from build123d import *

# Parameters (mm, degrees)
CHAMFER_1_SIZE           = 2
CUT_EXTRUDE_1_DEPTH      = 31
CUT_EXTRUDE_1_DEPTH_BACK = 20
SKETCH_2_W               = 91.624519514
SKETCH_2_H               = 25.767863676
HOLE_WIZARD_M10_1_D      = 8.5
HOLE_WIZARD_M10_1_DEPTH  = 27.5
HOLE_WIZARD_M10_1_TIP    = 2.553657631
CHAMFER_3_SIZE           = 1


with BuildPart() as part:
    # 草图1 → 旋转2 (revolve)
    with BuildSketch(Plane.XY):
        Polygon((0, 0), (0, 10), (23, 10), (23, 12.5), (120, 12.5), (120, 0), align=None)
    revolve(axis=Axis((120, 0, 0), (-1, 0, 0)))

    # 倒角1
    chamfer_1_edges = [part.edges().sort_by_distance(p)[0] for p in [
        (120, -12.5, 0),
        (0, -10, 0),
    ]]
    chamfer(chamfer_1_edges, length=CHAMFER_1_SIZE)

    # 草图2 → 切除-拉伸1 (cut, two sides: drawn at the far end of the back side and taken through both)
    with BuildSketch(Plane(origin=(0, 0, 0), x_dir=(1, 0, 0), z_dir=(0, 1, 0)).offset(-CUT_EXTRUDE_1_DEPTH_BACK)):
        with Locations((80.812259757, -17.883931838)):
            Rectangle(SKETCH_2_W, SKETCH_2_H)
    extrude(amount=CUT_EXTRUDE_1_DEPTH + CUT_EXTRUDE_1_DEPTH_BACK, mode=Mode.SUBTRACT)

    # M10 螺纹孔1
    with Locations(Plane.XY.offset(5)):
        with Locations((61, 0), (101, 0)):
            Hole(HOLE_WIZARD_M10_1_D / 2, depth=HOLE_WIZARD_M10_1_DEPTH)
            with Locations((0, 0, -(HOLE_WIZARD_M10_1_DEPTH + HOLE_WIZARD_M10_1_TIP / 2))):  # 118° drill point
                Cone(0, HOLE_WIZARD_M10_1_D / 2, HOLE_WIZARD_M10_1_TIP, mode=Mode.SUBTRACT)

    # 倒角3
    chamfer_3_edges = [part.edges().sort_by_distance(p)[0] for p in [
        (105.25, 0, 5),
        (65.25, 0, 5),
    ]]
    chamfer(chamfer_3_edges, length=CHAMFER_3_SIZE)


solid = part.part
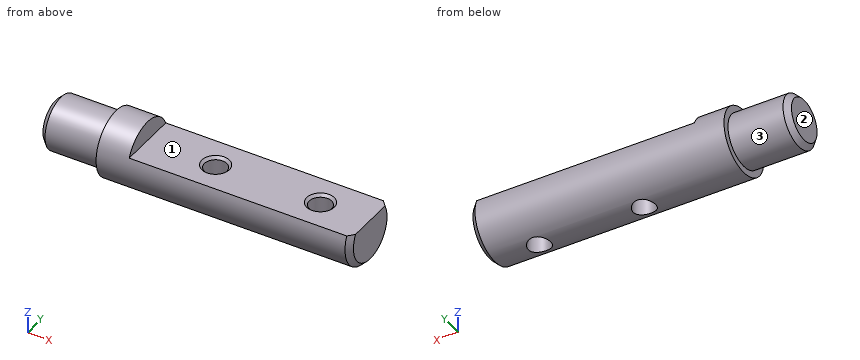
Design review of the part built by this model. Coordinates are the model's own, in mm. Face numbers are marked on the shaded views. Round coordinates to 2 decimals unless told otherwise and drop trailing zeros. Write each loop counter-clockwise with the first axis right and the second up, starting at its lowest first coordinate (ties: lowest second). Pieces come first, ordered by that corner, then holes. Notation, with made-up numbers: (-1, 15) - (28, 15) arc R30 ccw to (28, 46) - close; hole circle Ø2 at (62, 6). An arc over 180 degrees is marked (long way). Return JSON: item names as keys, results as strings. Group by question number.
Item 1: We need section D-D on x = 37.5. Write out the cut boundary in (y, z), and give its area (3 significant figures).
Item 2: We need section C-C on x = 61. Write out the cut boundary in (y, z).
Item 3: We need section B-B on y = 0. Write out the cut boundary in (x, z).
Item 4: The part is to be moulded in two halves that separate along Z. For the marked faces 1, 2 and 3, say which applies: pulls with the +Z half, pulls with the -Z half, needs draft (parallel to the pull), parting line crosses it, or undercut.
Item 5: We need section A-A on z = 0. Write out the cut boundary in (x, y).
Item 6: For probe 1 along X at (y, z) = (0, -5); probe 2 along Y at (x, z) = (101, -7.5); probe 3 along X at (y, z) = (-3.5, -2.75), list the stretches that pass through material, from the lowest coordinate up. Write a range as [from, to].
Item 7: Insertion check: P1, Ø1.5, axis at x = 101.5, y = 3, coming from the -Z side; P2, Ø6, axis at x = 51.5, y = -7, coming from the -Z side; P3, Ø11, axis at x = 61, y = 0, coming from the +Z side; P4, Ø12, axis at x = 85.5, z = -5, coming from the -Y side. Each pin has a flat end and moves straight along its axis. Give the tip position at first contact, or say it passes through.
Model answer:
{
 "1": {"outline": "(-11.46, 5) arc R12.5 ccw (long way) to (11.46, 5) - close", "area": "367 mm²"},
 "2": {"outline": "(-11.46, 5) arc R12.5 ccw to (-4.25, -11.76) - (-4.25, 4) - (-5.25, 5) - close; (4.25, -11.76) arc R12.5 ccw to (11.46, 5) - (5.25, 5) - (4.25, 4) - close"},
 "3": {"outline": "(0, -8) - (2, -10) - (23, -10) - (23, -12.5) - (56.75, -12.5) - (56.75, 4) - (55.75, 5) - (35, 5) - (35, 12.5) - (23, 12.5) - (23, 10) - (2, 10) - (0, 8) - close; (65.25, -12.5) - (96.75, -12.5) - (96.75, 4) - (95.75, 5) - (66.25, 5) - (65.25, 4) - close; (105.25, -12.5) - (118, -12.5) - (120, -10.5) - (120, 5) - (106.25, 5) - (105.25, 4) - close"},
 "4": {"face 1": "pulls with the +Z half", "face 2": "needs draft", "face 3": "parting line crosses it"},
 "5": {"outline": "(0, -8) - (2, -10) - (23, -10) - (23, -12.5) - (118, -12.5) - (120, -10.5) - (120, 10.5) - (118, 12.5) - (23, 12.5) - (23, 10) - (2, 10) - (0, 8) - close; hole circle Ø8.5 at (61, 0); hole circle Ø8.5 at (101, 0)"},
 "6": {"probe 1": "x = [0, 56.75], [65.25, 96.75], [105.25, 120]", "probe 2": "y = [-10, -4.25], [4.25, 10]", "probe 3": "x = [0, 58.59], [63.41, 98.59], [103.41, 120]"},
 "7": {"P1": "passes through", "P2": "stops at z = -11.84", "P3": "stops at z = 5", "P4": "stops at y = -12.5"}
}
